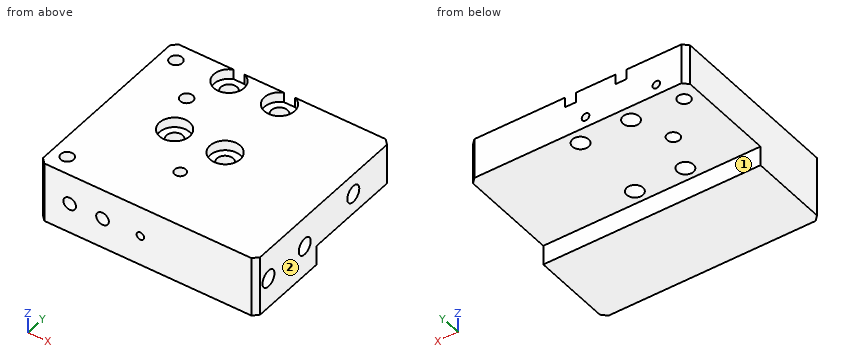
from build123d import *

# Parameters (mm, degrees)
SKETCH_1_W              = 40
SKETCH_1_H              = 27
EXTRUDE_1_DEPTH         = 6
SKETCH_2_R              = 1.1
CUT_EXTRUDE_1_DEPTH     = 10
MOVE_FACE_1_BY          = 10
SKETCH_3_W              = 3.9
SKETCH_3_H              = 20.4
CUT_EXTRUDE_2_DEPTH     = 63
HOLE_WIZARD_3_2_3_2_1_D = 3.2
MOVE_FACE_3_BY          = 3
HOLE_WIZARD_M4_2_D      = 3.3
HOLE_WIZARD_M4_2_DEPTH  = 11.5
HOLE_WIZARD_M4_2_TIP    = 0.991420021
SKETCH_16_R             = 3
CUT_EXTRUDE_3_DEPTH     = 2
HOLE_WIZARD_M3_1_D      = 2.5
HOLE_WIZARD_M3_1_DEPTH  = 8.5
HOLE_WIZARD_M3_1_TIP    = 0.751075774
CHAMFER_1_SIZE          = 1
SKETCH_20_R             = 0.75
CUT_EXTRUDE_4_DEPTH     = 66
PATTERN_LINEAR_1_COUNT  = 2
PATTERN_LINEAR_1_PITCH  = 14
HOLE_WIZARD_M3_2_D      = 2.5
HOLE_WIZARD_M3_3_D      = 2.5
HOLE_WIZARD_M3_3_DEPTH  = 8.5
HOLE_WIZARD_M3_3_TIP    = 0.751075774
HOLE_WIZARD_M4_3_D      = 3.3
HOLE_WIZARD_M4_3_DEPTH  = 11.5
HOLE_WIZARD_M4_3_TIP    = 0.991420021


with BuildPart() as part:
    # 草图1 → 凸台-拉伸1 (new, symmetric)
    with BuildSketch(Plane.XY):
        Rectangle(SKETCH_1_W, SKETCH_1_H)
    extrude(amount=EXTRUDE_1_DEPTH, both=True)

    # 草图2 → 切除-拉伸1 (cut)
    with BuildSketch(Plane.XY.offset(6)):
        with Locations((0, -2.5)):
            Circle(SKETCH_2_R)
    extrude(amount=-CUT_EXTRUDE_1_DEPTH, mode=Mode.SUBTRACT)

    # Move Face 1: a face moved outward by 10.0
    extrude(part.faces().sort_by_distance((0, 13.5, 0))[0], amount=MOVE_FACE_1_BY, dir=(0, 1, 0))

    # 草图3 → 切除-拉伸2 (cut)
    with BuildSketch(Plane(origin=(20, 0, 0), x_dir=(0, 0, -1), z_dir=(1, 0, 0))):
        with Locations((4.05, 13.3)):
            Rectangle(SKETCH_3_W, SKETCH_3_H)
    extrude(amount=-CUT_EXTRUDE_2_DEPTH, mode=Mode.SUBTRACT)

    # Ø3.2 (3.2) 直径孔1 (through all)
    with Locations(Plane.XY.offset(6)):
        with Locations((3, 20.7), (-7, 20.7), (-7, 5.7), (3, 5.7)):
            Hole(HOLE_WIZARD_3_2_3_2_1_D / 2)

    # Move Face 3: a face moved outward by 3.0
    extrude(part.faces().sort_by_distance((20, 3.188047415, 0.884145538))[0], amount=MOVE_FACE_3_BY, dir=(1, 0, 0))

    # M4 螺纹孔2
    with Locations(Plane(origin=(23, 0, 0), x_dir=(0, 0, -1), z_dir=(1, 0, 0))):
        with Locations((0, -0.2), (0, -10.2)):
            Hole(HOLE_WIZARD_M4_2_D / 2, depth=HOLE_WIZARD_M4_2_DEPTH)
            with Locations((0, 0, -(HOLE_WIZARD_M4_2_DEPTH + HOLE_WIZARD_M4_2_TIP / 2))):  # 118° drill point
                Cone(0, HOLE_WIZARD_M4_2_D / 2, HOLE_WIZARD_M4_2_TIP, mode=Mode.SUBTRACT)

    # 草图16 → 切除-拉伸3 (cut)
    with BuildSketch(Plane.XY.offset(6)):
        with Locations((-7, 20.7)):
            Circle(SKETCH_16_R)
        with Locations((3, 20.7)):
            Circle(SKETCH_16_R)
        with Locations((-7, 5.7)):
            Circle(SKETCH_16_R)
        with Locations((3, 5.7)):
            Circle(SKETCH_16_R)
    extrude(amount=-CUT_EXTRUDE_3_DEPTH, mode=Mode.SUBTRACT)

    # M3 螺纹孔1
    with Locations(Plane.XY.offset(6)):
        with Locations((-17, 20), (-17, -10)):
            Hole(HOLE_WIZARD_M3_1_D / 2, depth=HOLE_WIZARD_M3_1_DEPTH)
            with Locations((0, 0, -(HOLE_WIZARD_M3_1_DEPTH + HOLE_WIZARD_M3_1_TIP / 2))):  # 118° drill point
                Cone(0, HOLE_WIZARD_M3_1_D / 2, HOLE_WIZARD_M3_1_TIP, mode=Mode.SUBTRACT)

    # 倒角1
    chamfer_1_edges = [part.edges().sort_by_distance(p)[0] for p in [
        (23, -13.5, 0),
        (-20, -13.5, 0),
        (-20, 23.5, 1.95),
        (23, 23.5, 1.95),
    ]]
    chamfer(chamfer_1_edges, length=CHAMFER_1_SIZE)

    # 草图20 → 切除-拉伸4 (cut)
    with BuildSketch(Plane.XZ.offset(13.5)):
        with Locations(Location((0, 0, 0), (0, 0, 270))):
            Circle(SKETCH_20_R)
    cut_extrude_4 = extrude(amount=-CUT_EXTRUDE_4_DEPTH, mode=Mode.SUBTRACT)

    # 阵列(线性)1: 切除-拉伸4 ×2
    with Locations(*[(-i * PATTERN_LINEAR_1_PITCH, 0, 0) for i in range(1, PATTERN_LINEAR_1_COUNT)]):
        add(cut_extrude_4, mode=Mode.SUBTRACT)

    # M3 螺纹孔2 (through all)
    with Locations(Plane.XY.offset(6)):
        with Locations((-10, 13.2)):
            Hole(HOLE_WIZARD_M3_2_D / 2)

    # M3 螺纹孔3
    with Locations(Plane(origin=(0, -13.5, 0), x_dir=(-1, 0, 0), z_dir=(0, -1, 0))):
        with Locations((7.5, 0), (14, 0)):
            Hole(HOLE_WIZARD_M3_3_D / 2, depth=HOLE_WIZARD_M3_3_DEPTH)
            with Locations((0, 0, -(HOLE_WIZARD_M3_3_DEPTH + HOLE_WIZARD_M3_3_TIP / 2))):  # 118° drill point
                Cone(0, HOLE_WIZARD_M3_3_D / 2, HOLE_WIZARD_M3_3_TIP, mode=Mode.SUBTRACT)

    # M4 螺纹孔3
    with Locations(Plane(origin=(23, 0, 0), x_dir=(0, 0, -1), z_dir=(1, 0, 0))):
        with Locations((-1.95, 13.2)):
            Hole(HOLE_WIZARD_M4_3_D / 2, depth=HOLE_WIZARD_M4_3_DEPTH)
            with Locations((0, 0, -(HOLE_WIZARD_M4_3_DEPTH + HOLE_WIZARD_M4_3_TIP / 2))):  # 118° drill point
                Cone(0, HOLE_WIZARD_M4_3_D / 2, HOLE_WIZARD_M4_3_TIP, mode=Mode.SUBTRACT)


solid = part.part
Design review of the part built by this model. Coordinates are the model's own, in mm. Face numbers are marked on the shaded views. A direction names the side the tool comes from. Give positions to 0.01 mm unless a question says otherwise; leave off trailing zeros. Loops run counter-clockwise (first coordinate to the right, second up) from the corner with the lowest first, then second, coordinate; pieces in that order, holes last. Notation, with made-up numbers: M 84,63 L 119,63 A23 cw 119,99 Z; hole C -23,56.5 d10. An arc over 180 degrees is marked long. Answer as a JSON object with one key per item and string values.
Item 1: For P1, Ø3, axis at x = 3.5, y = 4.5, coming from the +Z side; P2, Ø6, axis at x = 6.5, y = 17, coming from the -Z side; P3, Ø1.5, axis at x = -7.5, z = 0, coming from the -Y side; P4, Ø1.4, axis at x = 0, z = 0, coming from the -Y side, all flat-tipped, find the tip position at first contact; note any pin that passes through.
Output values:
{"P1": "stops at z = 4", "P2": "stops at z = -2.1", "P3": "stops at y = -4.7", "P4": "passes through"}
Item 2: We need section D-D (z = -4.75). State the section outline as (x, y) points.
Output values:
{"outline": "M -20,-12.5 L -19,-13.5 L 22,-13.5 L 23,-12.5 L 23,3.1 L -20,3.1 Z"}
Item 3: Machinability: for the marked faces 1 and 2, which of the approach directions +Z, -Z, +X, -X, +Y, -Y give a long, thin tool a straight path to every point of the face, cutting with its end or side? Answer none if there is none.
Output values:
{"face 1": "-Z, +X, -X, +Y", "face 2": "+Z, -Z, +X, +Y, -Y"}
Item 4: Wall thickness on line 1 along Y through (x, z) = (-7, 2.5); line 2 along Y through (x, z) = (18.5, -0.5); line 3 along X through (y, z) = (20.7, 5.55): over which ranges is each line inside the solid? List them lowest first.
Output values:
{"line 1": "y = -13.5 to 4.1, 7.3 to 19.1, 22.3 to 23.5", "line 2": "y = -13.5 to -11.77, -8.63 to -1.77, 1.37 to 23.5", "line 3": "x = -20 to -18.04, -15.96 to -10, -4 to 0, 6 to 23"}
Item 5: We need section B-B (x = -14). State the section outline as (y, z) points.
Output values:
{"outline": "M -13.5,-6 L 3.1,-6 L 3.1,-2.1 L 23.5,-2.1 L 23.5,-0.75 L -4.7,-0.75 L -5,-1.25 L -13.5,-1.25 Z; M -13.5,1.25 L -5,1.25 L -4.7,0.75 L 23.5,0.75 L 23.5,6 L -13.5,6 Z"}
Item 6: We need section C-C (y = -2.5). State the section outline as (x, z) points.
Output values:
{"outline": "M -20,-6 L 23,-6 L 23,6 L 1.1,6 L 1.1,-4 L -1.1,-4 L -1.1,6 L -20,6 Z; hole C -14,0 d1.5"}
Item 7: We need section A-A (y = 5.7). State the section outline as (x, z) points.
Output values:
{"outline": "M -20,-2.1 L -8.6,-2.1 L -8.6,4 L -10,4 L -10,6 L -20,6 Z; M -5.4,-2.1 L 1.4,-2.1 L 1.4,4 L 0,4 L 0,6 L -4,6 L -4,4 L -5.4,4 Z; M 4.6,-2.1 L 23,-2.1 L 23,6 L 6,6 L 6,4 L 4.6,4 Z; hole C -14,0 d1.5; hole C 0,0 d1.5"}
